from build123d import *

# Parameters (mm, degrees)
SKETCH_1_R      = 11
SKETCH_1_R_2    = 9
EXTRUDE_1_DEPTH = 6
SKETCH_2_R      = 11
SKETCH_2_R_2    = 2.6
EXTRUDE_2_DEPTH = 2
CHAMFER_1_SIZE  = 1
EXTRUDE_START   = -2
SKETCH_3_R      = 17
SKETCH_3_R_2    = 9
EXTRUDE_3_DEPTH = 2
CHAMFER_2_SIZE  = 1


with BuildPart() as part:
    # 草图1 → 凸台-拉伸1 (new body)
    with BuildSketch(Plane.XY):
        Circle(SKETCH_1_R)
        Circle(SKETCH_1_R_2, mode=Mode.SUBTRACT)
    extrude(amount=EXTRUDE_1_DEPTH)

    # 草图2 → 凸台-拉伸2 (add)
    with BuildSketch(Plane(origin=(0, 0, 0), x_dir=(-1, 0, 0), z_dir=(0, 0, -1))):
        with Locations(Location((0, 0, 0), (0, 0, 180))):
            Circle(SKETCH_2_R)
        Circle(SKETCH_2_R_2, mode=Mode.SUBTRACT)
    extrude(amount=-EXTRUDE_2_DEPTH)

    # 倒角1
    chamfer_1_edges = [part.edges().sort_by_distance(p)[0] for p in [
        (-9, 0, 2),
        (-11, 0, 0),
    ]]
    chamfer(chamfer_1_edges, length=CHAMFER_1_SIZE)

    # 草图3 → 凸台-拉伸3 (add)
    with BuildSketch(Plane.XY.offset(6).offset(EXTRUDE_START)):
        Circle(SKETCH_3_R)
        with Locations(Location((0, 0, 0), (0, 0, 180))):
            Circle(SKETCH_3_R_2, mode=Mode.SUBTRACT)
    extrude(amount=EXTRUDE_3_DEPTH)

    # 倒角2
    chamfer_2_edges = [part.edges().sort_by_distance(p)[0] for p in [
        (-17, 0, 6),
        (-9, 0, 6),
    ]]
    chamfer(chamfer_2_edges, length=CHAMFER_2_SIZE)


solid = part.part
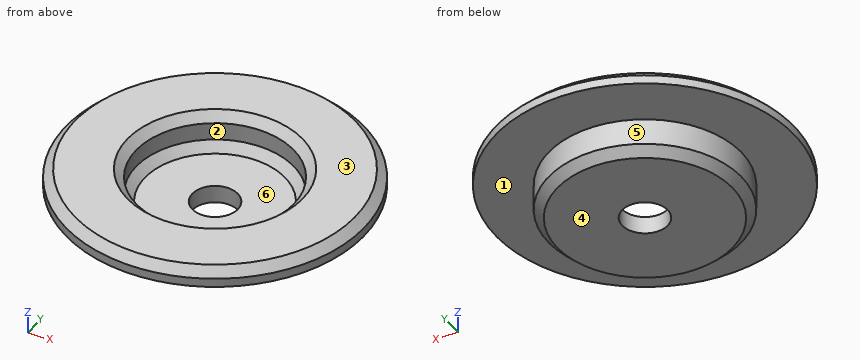
The model under review builds one solid part; all positions refer to its coordinate system, in mm. Face numbers are marked on the shaded views. A direction names the side the tool comes from. Round coordinates to 2 decimals unless told otherwise and drop trailing zeros. Loops run counter-clockwise (first coordinate to the right, second up) from the corner with the lowest first, then second, coordinate; pieces in that order, holes last. Notation, with made-up numbers: (-38, -29) - (15, -29) arc R27 ccw to (15, -13) - close; hole circle Ø11 at (9.5, -29). An arc over 180 degrees is marked (long way). Use CSV: the item, a comma, the result in double quotes.
(1) The part is to be moulded in two halves that separate along X. For the marked faces 4, 5 and 6, say which applies: pulls with the +X half, pulls with the -X half, needs draft (parallel to the pull), parting line crosses it, or undercut.
Working result:
face 4,"needs draft"
face 5,"parting line crosses it"
face 6,"undercut"
(2) Clearance check with flat-ended pins moving along their axes: P1, Ø2, axis at y = -6, z = 0.5, coming from the -X side; P2, Ø5, axis at x = -1, y = -1.5, coming from the +Z side; P3, Ø1, axis at y = -12.5, z = 4, coming from the +X side. State where each tip first meets the part, or that it passes through.
Working result:
P1,"stops at x = -9.73"
P2,"stops at z = 2"
P3,"stops at x = 12.04"
(3) Machinability: for the marked faces 1, 2 and 3, which of the approach directions +Z, -Z, +X, -X, +Y, -Y give a long, thin tool a straight path to every point of the face, cutting with its end or side? Answer none if there is none.
Working result:
face 1,"-Z"
face 2,"+Z"
face 3,"+Z, +X, -X, +Y, -Y"
(4) Take a section at A-A, the plane y = 0. Give the boundary of the cut face in (x, z), plus the area to 3 significant figures.
Working result:
outline,"(-17, 4) - (-11, 4) - (-11, 1) - (-10, 0) - (-2.6, 0) - (-2.6, 2) - (-8, 2) - (-9, 3) - (-9, 5) - (-10, 6) - (-16, 6) - (-17, 5) - close; (2.6, 0) - (10, 0) - (11, 1) - (11, 4) - (17, 4) - (17, 5) - (16, 6) - (10, 6) - (9, 5) - (9, 3) - (8, 2) - (2.6, 2) - close"
area,"71.6 mm^2"
(5) For line 1 (Y direction, x = 0, z = 1.5); line 2 (Y direction, x = 0, z = 4.55); line 3 (Z direction, x = -4.5, y = 1), list the stretches that pass through material, from the lowest coordinate up.
Working result:
line 1,"y = -11 to -2.6, 2.6 to 11"
line 2,"y = -17 to -9, 9 to 17"
line 3,"z = 0 to 2"
